Build history of the part. All positions in model axes, mm. Round coordinates to 2 decimals unless told otherwise and drop trailing zeros. Order: outer loops, then holes, each group sorted by start corner. A loop starts at its lowest first (then second) coordinate and runs counter-clockwise, first axis right, second up. Notation, with made-up numbers: (7.25, 74) -> (63.25, 74) arc R27 ccw to (63.25, 113) -> close; hole circle Ø1 at (-36.75, 52.25). An arc over 180 degrees is marked (long way). Use a Markdown table: item, result. Add a question column.
Item 1: Slice it at A-A, the plane x = 765. Give the cut face in (y, z).
Item 2: Probe L1, parallel to X at y = 42.5, z = 13; L2, parallel to Y at x = 461, z = 19; L3, parallel to Y at x = 768, z = 30. List the from-to ranges inside material, lowest first.
Item 3: Pin check, flat tip, straight feed: pin 1 (12 mm diameter, centred on x = 509, z = 6.5, fed in from -Y). Stop position of the tip, or through.
Item 4: Slice it at B-B, the plane y = 40. Give the cut face in (x, z), plus the area to 3 significant figures.
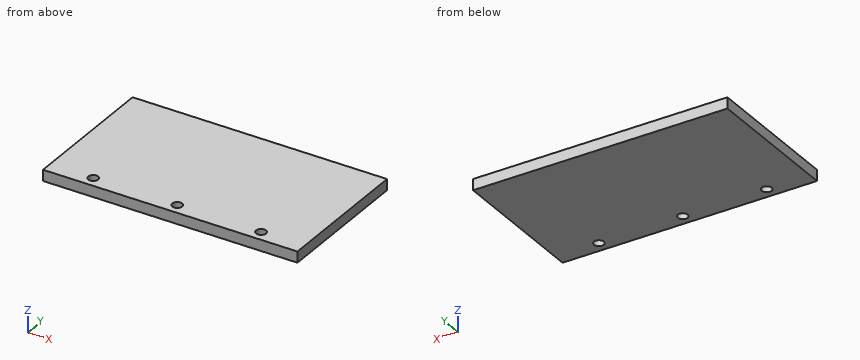
from build123d import *

# Parameters (mm, degrees)
SKETCH1_W           = 922
SKETCH1_H           = 515
SKETCH1_R           = 18
BOSS_EXTRUDE1_DEPTH = 40


with BuildPart() as part:
    # Sketch1 → Boss-Extrude1 (new body)
    with BuildSketch(Plane.XY):
        with Locations((461, 257.5)):
            Rectangle(SKETCH1_W, SKETCH1_H)
        with Locations((461, 40)):
            Circle(SKETCH1_R, mode=Mode.SUBTRACT)
        with Locations((765, 40)):
            Circle(SKETCH1_R, mode=Mode.SUBTRACT)
        with Locations((157, 40)):
            Circle(SKETCH1_R, mode=Mode.SUBTRACT)
    extrude(amount=BOSS_EXTRUDE1_DEPTH)


solid = part.part
Check sheet entries:
| question | item | result |
|---|---|---|
| 1 | outline | (0, 0) -> (22, 0) -> (22, 40) -> (0, 40) -> close; (58, 0) -> (515, 0) -> (515, 40) -> (58, 40) -> close |
| 2 | L1 | 0 to 139.17, 174.83 to 443.17, 478.83 to 747.17, 782.83 to 922 |
| 2 | L2 | 0 to 22, 58 to 515 |
| 2 | L3 | 0 to 22.25, 57.75 to 515 |
| 3 | pin 1 | y = 0 |
| 4 | outline | (0, 0) -> (139, 0) -> (139, 40) -> (0, 40) -> close; (175, 0) -> (443, 0) -> (443, 40) -> (175, 40) -> close; (479, 0) -> (747, 0) -> (747, 40) -> (479, 40) -> close; (783, 0) -> (922, 0) -> (922, 40) -> (783, 40) -> close |
| 4 | area | 32,600 mm2 |
